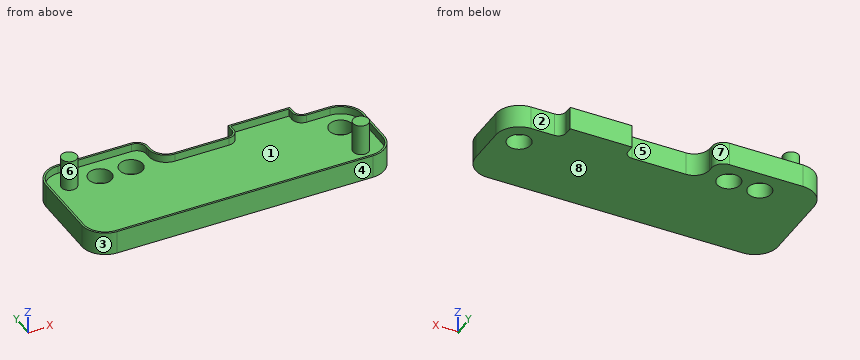
```python
from build123d import *

# Parameters (mm, degrees)
PLATE_OUTLINE_SKETCH_R       = 1
PLATE_OUTLINE_SKETCH_R_2     = 1.5
BASE_PLATE_3MM_DEPTH         = 3
RECESS_POCKET_1MM_DEPTH      = 22.106870919
RECESS_POCKET_1MM_DEPTH_BACK = 1
LOCATING_PIN_SKETCH_R        = 1
LOCATING_PINS_2X_DEPTH       = 6


with BuildPart() as part:
    # Plate Outline Sketch → Base Plate 3mm (new body)
    with BuildSketch(Plane.XY):
        with BuildLine():
            Line((4.5, 5.5), (12.5, 5.5))
            Line((12.5, 5.5), (12.5, 4.5))
            ThreePointArc((12.5, 4.5), (12.792893219, 3.792893219), (13.5, 3.5))
            Line((13.5, 3.5), (16.5, 3.5))
            ThreePointArc((16.5, 3.5), (18.621320344, 2.621320344), (19.5, 0.5))
            Line((19.5, 0.5), (19.5, -4.5))
            ThreePointArc((19.5, -4.5), (18.621320344, -6.621320344), (16.5, -7.5))
            Line((16.5, -7.5), (-16.5, -7.5))
            ThreePointArc((-16.5, -7.5), (-18.621320344, -6.621320344), (-19.5, -4.5))
            Line((-19.5, -4.5), (-19.5, 4.5))
            ThreePointArc((-19.5, 4.5), (-18.621320344, 6.621320344), (-16.5, 7.5))
            Line((-16.5, 7.5), (-7, 7.5))
            ThreePointArc((-7, 7.5), (-5.939339828, 7.060660172), (-5.5, 6))
            Line((-5.5, 6), (-5.5, 5.5))
            ThreePointArc((-5.5, 5.5), (-4.914213562, 4.085786438), (-3.5, 3.5))
            Line((-3.5, 3.5), (3.5, 3.5))
            ThreePointArc((3.5, 3.5), (4.207106781, 3.792893219), (4.5, 4.5))
            Line((4.5, 4.5), (4.5, 5.5))
        make_face()
        with Locations((-16.5, 4.5)):
            Circle(PLATE_OUTLINE_SKETCH_R, mode=Mode.SUBTRACT)
        with Locations((-12.5, 4.5)):
            Circle(PLATE_OUTLINE_SKETCH_R_2, mode=Mode.SUBTRACT)
        with Locations((-8.5, 4.5)):
            Circle(PLATE_OUTLINE_SKETCH_R_2, mode=Mode.SUBTRACT)
        with Locations((16.5, 0.5)):
            Circle(PLATE_OUTLINE_SKETCH_R_2, mode=Mode.SUBTRACT)
        with Locations((16.5, -4.5)):
            Circle(PLATE_OUTLINE_SKETCH_R, mode=Mode.SUBTRACT)
    extrude(amount=BASE_PLATE_3MM_DEPTH)

    # Pocket Outline Sketch → Recess Pocket 1mm (cut, two sides: drawn at the far end of the back side and taken through both)
    with BuildSketch(Plane.XY.offset(3).offset(-RECESS_POCKET_1MM_DEPTH_BACK)):
        with BuildLine():
            Line((16.5, 3.25), (13.5, 3.25))
            ThreePointArc((13.5, 3.25), (12.616116524, 3.616116524), (12.25, 4.5))
            Line((12.25, 4.5), (12.25, 5.25))
            Line((12.25, 5.25), (4.75, 5.25))
            Line((4.75, 5.25), (4.75, 4.5))
            ThreePointArc((4.75, 4.5), (4.383883476, 3.616116524), (3.5, 3.25))
            Line((3.5, 3.25), (-3.5, 3.25))
            ThreePointArc((-3.5, 3.25), (-5.090990258, 3.909009742), (-5.75, 5.5))
            Line((-5.75, 5.5), (-5.75, 6))
            ThreePointArc((-5.75, 6), (-6.116116524, 6.883883476), (-7, 7.25))
            Line((-7, 7.25), (-16.5, 7.25))
            ThreePointArc((-16.5, 7.25), (-18.444543648, 6.444543648), (-19.25, 4.5))
            Line((-19.25, 4.5), (-19.25, -4.5))
            ThreePointArc((-19.25, -4.5), (-18.444543648, -6.444543648), (-16.5, -7.25))
            Line((-16.5, -7.25), (16.5, -7.25))
            ThreePointArc((16.5, -7.25), (18.444543648, -6.444543648), (19.25, -4.5))
            Line((19.25, -4.5), (19.25, 0.5))
            ThreePointArc((19.25, 0.5), (18.444543648, 2.444543648), (16.5, 3.25))
        make_face()
    extrude(amount=RECESS_POCKET_1MM_DEPTH + RECESS_POCKET_1MM_DEPTH_BACK, mode=Mode.SUBTRACT)

    # Locating Pin Sketch → Locating Pins 2x (add)
    with BuildSketch(Plane(origin=(0, 0, 0), x_dir=(-1, 0, 0), z_dir=(0, 0, -1))):
        with Locations((16.5, 4.5)):
            Circle(LOCATING_PIN_SKETCH_R)
        with Locations((-16.5, -4.5)):
            Circle(LOCATING_PIN_SKETCH_R)
    extrude(amount=-LOCATING_PINS_2X_DEPTH)


solid = part.part
```
Build history of the part. All positions in model axes, mm. Face numbers are marked on the shaded views. A direction names the side the tool comes from. Give positions to 0.01 mm unless a question says otherwise; leave off trailing zeros. Loops run counter-clockwise (first coordinate to the right, second up) from the corner with the lowest first, then second, coordinate; pieces in that order, holes last.
Item 1: Which spindle directions (+Z, -Z, +X, -X, +Y, -Y) get a long thin tool onto all of the face, cutting with end or side? Do the marked faces 1, 2, 3, 4 and 5. Say none if no direction does.
Answers follow:
face 1: +Z
face 2: +Z, -Z, +X, +Y
face 3: +Z, -Z, -X, -Y
face 4: +Z, -Z, +X, -X, -Y
face 5: +Z, -Z, +Y
Item 2: Pull direction X, two halves, no side cores. Call the marked faces 6, 7 and 8: released by +X, released by -X, zero draft, split by the parting line, or undercut.
Answers follow:
face 6: undercut
face 7: released by +X
face 8: zero draft
Item 3: Drill centre lines: line 1 (Y direction, x = 16.5, z = 0.75); line 2 (Y direction, x = -1, z = 2.4); line 3 (X direction, y = 4.5, z = 1.5). Where is each one in solid material? Low to high.
Answers follow:
line 1: y = -7.5 to -1, 2 to 3.5
line 2: y = -7.5 to -7.25, 3.25 to 3.5
line 3: x = -19.5 to -14, -11 to -10, -7 to -5.23, 4.5 to 12.5
Item 4: Flat gauge pins, fed straight in: pin 1 (6 mm diameter, centred on x = -2, y = 3.5, fed in from +Z); pin 2 (4 mm diameter, centred on x = -12.5, y = 4.5, fed in from +Z); pin 3 (1 mm diameter, centred on y = 5.5, z = 4, fed in from -X); pin 4 (1.8 mm diameter, centred on x = 16.5, y = 0.5, fed in from +Z). Where does each tip first touch, or does it go through?
Answers follow:
pin 1: stops at z = 3
pin 2: stops at z = 2
pin 3: stops at x = -17.37
pin 4: passes through
Item 5: Slice it at D-D, the plane y = 1. List the corners of the cut face in (x, z).
Answers follow:
outline: (-19.5, 0) - (15.09, 0) - (15.09, 2) - (-19.25, 2) - (-19.25, 3) - (-19.5, 3) - close; (17.91, 0) - (19.46, 0) - (19.46, 3) - (19.2, 3) - (19.2, 2) - (17.91, 2) - close
Item 6: Slice it at A-A, the plane x = -8.5. List the corners of the cut face in (y, z), and give its area (3 significant figures).
Answers follow:
outline: (-7.5, 0) - (3, 0) - (3, 2) - (-7.25, 2) - (-7.25, 3) - (-7.5, 3) - close; (6, 0) - (7.5, 0) - (7.5, 3) - (7.25, 3) - (7.25, 2) - (6, 2) - close
area: 24.5 mm2
Item 7: Slice it at C-C, the plane x = 5.5. List the corners of the cut face in (y, z).
Answers follow:
outline: (-7.5, 0) - (5.5, 0) - (5.5, 3) - (5.25, 3) - (5.25, 2) - (-7.25, 2) - (-7.25, 3) - (-7.5, 3) - close
Item 8: Slice it at B-B, the plane z = 1.05. List the corners of the cut face in (x, y), and give its area (3 significant figures).
Answers follow:
outline: (-19.5, -4.5) arc R3 ccw to (-16.5, -7.5) - (16.5, -7.5) arc R3 ccw to (19.5, -4.5) - (19.5, 0.5) arc R3 ccw to (16.5, 3.5) - (13.5, 3.5) arc R1 cw to (12.5, 4.5) - (12.5, 5.5) - (4.5, 5.5) - (4.5, 4.5) arc R1 cw to (3.5, 3.5) - (-3.5, 3.5) arc R2 cw to (-5.5, 5.5) - (-5.5, 6) arc R1.5 ccw to (-7, 7.5) - (-16.5, 7.5) arc R3 ccw to (-19.5, 4.5) - close; hole circle Ø3 at (-12.5, 4.5); hole circle Ø3 at (-8.5, 4.5); hole circle Ø3 at (16.5, 0.5)
area: 473 mm2
